from build123d import *

# Parameters (mm, degrees)
EXTRUDE_1_DEPTH     = 36
SKETCH_2_R          = 3
EXTRUDE_2_DEPTH     = 14.5
SKETCH_3_R          = 1.55
SKETCH_3_R_2        = 2.05
CUT_EXTRUDE_1_DEPTH = 41.652921174
FILLET_1_R          = 3
FILLET_2_R          = 1


with BuildPart() as part:
    # 草图1 → 凸台-拉伸1 (new body)
    with BuildSketch(Plane.XY):
        Polygon((-6.1, 6), (6.1, 6), (6.1, -5.5), (9.1, -5.5), (9.1, 9), (-9.1, 9), (-9.1, -5.5), (-6.1, -5.5), align=None)
    extrude(amount=EXTRUDE_1_DEPTH)

    # 草图2 → 凸台-拉伸2 (add)
    with BuildSketch(Plane(origin=(0, 9, 0), x_dir=(1, 0, 0), z_dir=(0, 1, 0))):
        with Locations((9.1, -3)):
            Circle(SKETCH_2_R)
        with Locations((-9.1, -3)):
            Circle(SKETCH_2_R)
        with Locations((9.1, -33)):
            Circle(SKETCH_2_R)
        with Locations((-9.1, -33)):
            Circle(SKETCH_2_R)
    extrude(amount=-EXTRUDE_2_DEPTH)

    # 草图3 → 切除-拉伸1 (cut, through all)
    with BuildSketch(Plane(origin=(0, 9, 0), x_dir=(1, 0, 0), z_dir=(0, 1, 0))):
        with Locations(Location((9.1, -3, 0), (0, 0, 180))):
            Circle(SKETCH_3_R)
        with Locations(Location((-9.1, -33, 0), (0, 0, 180))):
            Circle(SKETCH_3_R)
        with Locations(Location((9.1, -33, 0), (0, 0, 180))):
            Circle(SKETCH_3_R)
        with Locations(Location((-9.1, -3, 0), (0, 0, 180))):
            Circle(SKETCH_3_R)
        with Locations(Location((0, -18, 0), (0, 0, 180))):
            Circle(SKETCH_3_R_2)
    extrude(amount=-CUT_EXTRUDE_1_DEPTH, mode=Mode.SUBTRACT)

    # 圆角1
    fillet_1_edges = [part.edges().sort_by_distance(p)[0] for p in [
        (9.1, 1.75, 6),
        (-9.1, 1.75, 6),
        (9.1, 1.75, 30),
        (-9.1, 1.75, 30),
    ]]
    fillet(fillet_1_edges, radius=FILLET_1_R)

    # 圆角2
    fillet_2_edges = [part.edges().sort_by_distance(p)[0] for p in [
        (6.1, 0.25, 0),
        (-6.1, 0.25, 0),
        (6.1, 0.25, 36),
        (-6.1, 0.25, 36),
    ]]
    fillet(fillet_2_edges, radius=FILLET_2_R)


solid = part.part
Here's how the part is built. I have some questions about the finished solid (model axes, mm). A direction names the side the tool comes from. Round coordinates to 2 decimals unless told otherwise and drop trailing zeros. Write each loop counter-clockwise with the first axis right and the second up, starting at its lowest first coordinate (ties: lowest second). Pieces come first, ordered by that corner, then holes. Notation, with made-up numbers: (63.5, 1.25) -> (122.5, 1.25) arc R17 ccw to (122.5, 20.25) -> close; hole circle Ø6 at (58, -18.5). An arc over 180 degrees is marked (long way). One line per item, written item: value.
1) Suppose I cut it at A-A on y = 1.5. List the corners of the cut face in (x, z) for me, plus the area to 3 significant figures.
Filled sheet:
outline: (-10.6, 5.6) arc R3 ccw to (-9.1, 0) -> (-7.1, 0) arc R1 ccw to (-6.1, 1) -> (-6.1, 35) arc R1 ccw to (-7.1, 36) -> (-9.1, 36) arc R3 ccw to (-10.6, 30.4) arc R3 cw to (-9.1, 27.8) -> (-9.1, 8.2) arc R3 cw to start; (6.1, 1) arc R1 ccw to (7.1, 0) -> (9.1, 0) arc R3 ccw to (10.6, 5.6) arc R3 cw to (9.1, 8.2) -> (9.1, 27.8) arc R3 cw to (10.6, 30.4) arc R3 ccw to (9.1, 36) -> (7.1, 36) arc R1 ccw to (6.1, 35) -> close; hole circle Ø3.1 at (-9.1, 3); hole circle Ø3.1 at (-9.1, 33); hole circle Ø3.1 at (9.1, 3); hole circle Ø3.1 at (9.1, 33)
area: 244 mm2
2) If I drill on line 1 (X direction, y = -3, z = 22); line 2 (X direction, y = -4.25, z = 2); line 3 (Y direction, x = 1.5, z = 32.5), over which ranges is the centre line in solid material (lowest first)? Write a range as [from, to].
Filled sheet:
line 1: x = [-9.1, -6.1], [6.1, 9.1]
line 2: x = [-11.93, -10.28], [-7.92, -6.1], [6.1, 7.92], [10.28, 11.93]
line 3: y = [6, 9]
3) For faces 5 (the face through (6.401, 0.17, 35.715)), 6 (the face through (-9.1, 2, 18)), 7 (the face through (-6.1, 0, 18)), which set-ups out of +Z, -Z, +X, -X, +Y, -Y let a thin tool reach every point of the face, with its end or its side?
Filled sheet:
face 5: +Z, -Y
face 6: -X, +Y, -Y
face 7: +Z, -Z, -Y
4) Suppose I cut it at D-D on x = 0. List the corners of the cut face in (y, z) for me.
Filled sheet:
outline: (6, 0) -> (9, 0) -> (9, 15.95) -> (6, 15.95) -> close; (6, 20.05) -> (9, 20.05) -> (9, 36) -> (6, 36) -> close
5) Suppose I cut it at C-C on y = 8.25. List the corners of the cut face in (x, z) for me.
Filled sheet:
outline: (-10.6, 5.6) arc R3 ccw to (-9.1, 0) -> (9.1, 0) arc R3 ccw to (10.6, 5.6) arc R3 cw to (9.1, 8.2) -> (9.1, 27.8) arc R3 cw to (10.6, 30.4) arc R3 ccw to (9.1, 36) -> (-9.1, 36) arc R3 ccw to (-10.6, 30.4) arc R3 cw to (-9.1, 27.8) -> (-9.1, 8.2) arc R3 cw to start; hole circle Ø3.1 at (-9.1, 3); hole circle Ø3.1 at (-9.1, 33); hole circle Ø4.1 at (0, 18); hole circle Ø3.1 at (9.1, 3); hole circle Ø3.1 at (9.1, 33)
6) I'm going to push flat-ended pins straight in: pin 1 Ø3.5 at (x, z) = (0, 18) entering from +Y; pin 2 Ø8 at (x, z) = (1.5, 12) entering from -Y; pin 3 Ø3 at (y, z) = (3.5, 21.5) entering from +X. Where does each tip first touch, or does it pass through?
Filled sheet:
pin 1: passes through
pin 2: stops at y = 6
pin 3: stops at x = 9.1
7) Suppose I cut it at B-B on z = 3. List the corners of the cut face in (x, y) for me.
Filled sheet:
outline: (-12.1, -5.5) -> (-10.65, -5.5) -> (-10.65, 9) -> (-12.1, 9) -> close; (-7.55, -5.5) -> (-6.1, -5.5) -> (-6.1, 6) -> (6.1, 6) -> (6.1, -5.5) -> (7.55, -5.5) -> (7.55, 9) -> (-7.55, 9) -> close; (10.65, -5.5) -> (12.1, -5.5) -> (12.1, 9) -> (10.65, 9) -> close
8) We'd pull the mould along Z, two halves only. Please class faces 1 (the face through (10.33, 1.85, 2.06)), 2 (the face through (-6.401, 0.33, 35.715)), 3 (the face through (-8, -5.5, 18)), 4 (the face through (0, 7, 0)): released by +Z, released by -Z, zero draft, split by the parting line, or undercut.
Filled sheet:
face 1: undercut
face 2: released by +Z
face 3: zero draft
face 4: released by -Z
